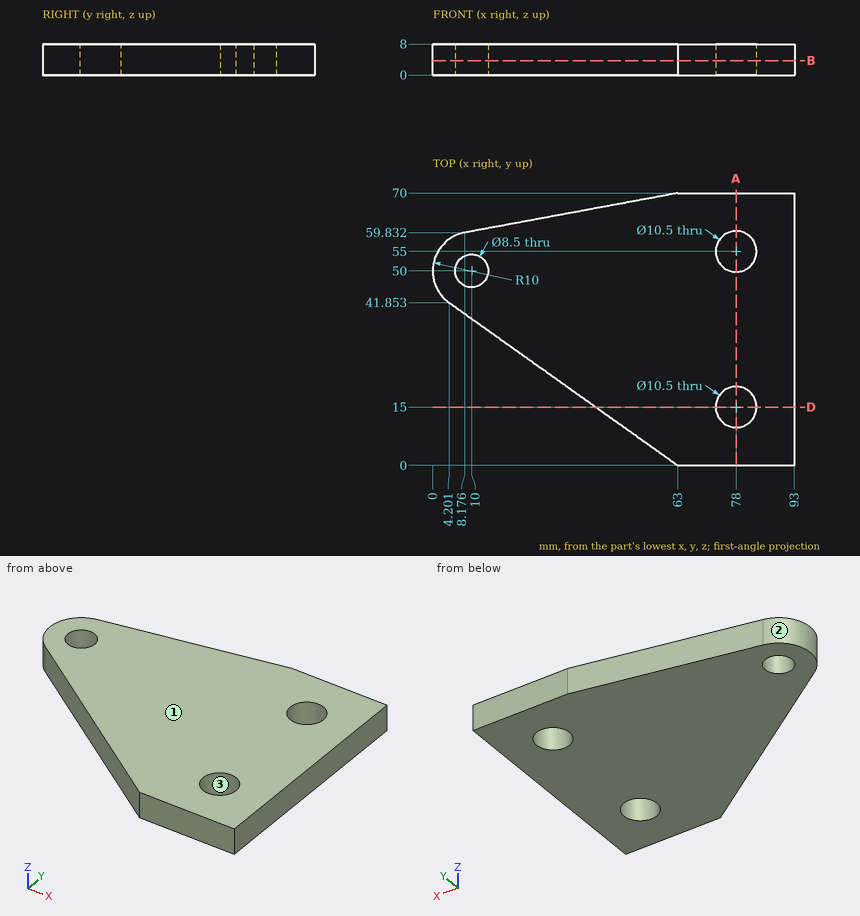
Could you check a few things on this drawing? It's one solid part, dimensions in mm from its lowest x, y, z. Round coordinates to 2 decimals unless told otherwise and drop trailing zeros. Order: outer loops, then holes, each group sorted by start corner. A loop starts at its lowest first (then second) coordinate and runs counter-clockwise, first axis right, second up.
Q1. I'm going to push a flat-ended pin straight in: P1, Ø4, axis at x = 58, z = 2.5, coming from the +Y side. Where does the tip first touch, or does it pass through?
Geometry says:
P1: stops at y = 69.44
Q2. Imagine slicing it at B-B, the plane z = 3.75. List the corners of the cut face in (x, y) for me, then the cut area to 3 significant figures.
Geometry says:
outline: (4.2, 41.85) - (63, 0) - (93, 0) - (93, 70) - (63, 70) - (8.18, 59.83) arc R10 ccw to start; hole circle Ø8.5 at (10, 50); hole circle Ø10.5 at (78, 15); hole circle Ø10.5 at (78, 55)
area: 4,480 mm2
Q3. Thinking about a two-plate mould opening in X: for the marked faces 1, 2 and 3, which applies, released by +X, released by -X, zero draft, split by the parting line, or undercut?
Geometry says:
face 1: zero draft
face 2: released by -X
face 3: undercut
Q4. Please list where these lines run through material, in increasing order: probe 1 along Y at (x, z) = (78, 3.75); probe 2 along X at (y, z) = (55, 3); probe 3 along Y at (x, z) = (9.5, 3).
Geometry says:
probe 1: y = 0 to 9.75, 20.25 to 49.75, 60.25 to 70
probe 2: x = 1.34 to 72.75, 83.25 to 93
probe 3: y = 38.08 to 45.78, 54.22 to 60.08
Q5. Imagine slicing it at A-A, the plane x = 78. List the corners of the cut face in (y, z) for me.
Geometry says:
outline: (0, 0) - (9.75, 0) - (9.75, 8) - (0, 8) - close; (20.25, 0) - (49.75, 0) - (49.75, 8) - (20.25, 8) - close; (60.25, 0) - (70, 0) - (70, 8) - (60.25, 8) - close
Q6. Imagine slicing it at D-D, the plane y = 15. List the corners of the cut face in (x, z) for me.
Geometry says:
outline: (41.93, 0) - (72.75, 0) - (72.75, 8) - (41.93, 8) - close; (83.25, 0) - (93, 0) - (93, 8) - (83.25, 8) - close
